```python
from build123d import *

# Parameters (mm, degrees)
SKETCH1_R                = 50
BOSS_EXTRUDE1_DEPTH      = 5
SKETCH2_R                = 15
BOSS_EXTRUDE2_DEPTH      = 5
SKETCH3_R                = 9
CUT_EXTRUDE1_DEPTH       = 15
BOSS_EXTRUDE3_REACH      = 118.726
BOSS_EXTRUDE3_END_RADIUS = 50
SKETCH6_R                = 1.25
BOSS_EXTRUDE4_DEPTH      = 5
CIRPATTERN3_COUNT        = 4


with BuildPart() as part:
    # Sketch1 → Boss-Extrude1 (new body)
    with BuildSketch(Plane.XY):
        Circle(SKETCH1_R)
    extrude(amount=BOSS_EXTRUDE1_DEPTH)

    # Sketch2 → Boss-Extrude2 (add)
    with BuildSketch(Plane.XY.offset(5)):
        Circle(SKETCH2_R)
    extrude(amount=BOSS_EXTRUDE2_DEPTH)

    # Sketch3 → Cut-Extrude1 (cut)
    with BuildSketch(Plane.XY.offset(10)):
        Circle(SKETCH3_R)
    extrude(amount=-CUT_EXTRUDE1_DEPTH, mode=Mode.SUBTRACT)

    # Boss-Extrude3: up to this cylinder (the profile starts outside it)
    boss_extrude3_end = Plane(origin=(0, 0, 2.5), z_dir=(0, 0, -1)) * Cylinder(BOSS_EXTRUDE3_END_RADIUS, 338.452, mode=Mode.PRIVATE)
    # Sketch4 → Boss-Extrude3 (add, up to the surface)
    with BuildSketch(Plane(origin=(0, 55, 0), x_dir=(1, 0, 0), z_dir=(0, 1, 0)), mode=Mode.PRIVATE) as boss_extrude3_sk1:
        Polygon((0, 0), (2.5, 0), (2.5, -5), (-2.5, -5), (-2.5, 0), align=None)
    boss_extrude3_tool1 = extrude(boss_extrude3_sk1.sketch, amount=-BOSS_EXTRUDE3_REACH, mode=Mode.PRIVATE) - boss_extrude3_end
    boss_extrude3 = boss_extrude3_tool1.solids().sort_by_distance((0, 55, 2.5))[0]
    add(boss_extrude3)

    # Sketch6 → Boss-Extrude4 (add, symmetric)
    with BuildSketch(Plane(origin=(0, 0, 0), x_dir=(0, 0, -1), z_dir=(1, 0, 0))):
        with Locations(Location((-2.5, 52.8, 0), (0, 0, 180))):
            Circle(SKETCH6_R)
    boss_extrude4 = extrude(amount=BOSS_EXTRUDE4_DEPTH, both=True)

    # CirPattern3: Boss-Extrude3, Boss-Extrude4 ×4 about axis
    cirpattern3_axis = Axis((0, 0, 0), (0, 0, 1))
    add([boss_extrude3.rotate(cirpattern3_axis, i * 360 / CIRPATTERN3_COUNT) for i in range(1, CIRPATTERN3_COUNT)])
    add([boss_extrude4.rotate(cirpattern3_axis, i * 360 / CIRPATTERN3_COUNT) for i in range(1, CIRPATTERN3_COUNT)])


solid = part.part
```
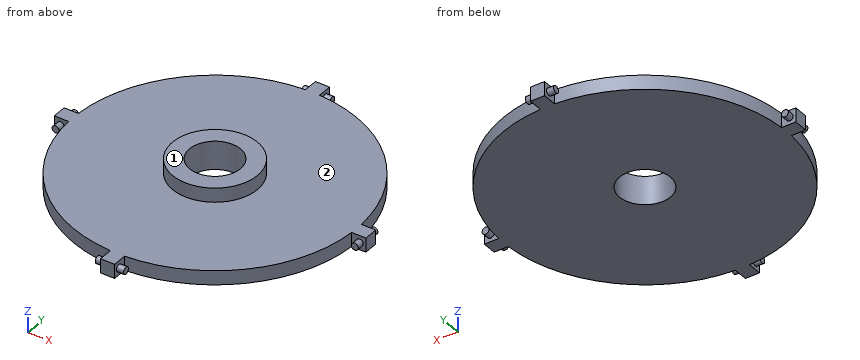
Verification items for the finished model (mm, model axes). Face numbers are marked on the shaded views. A direction names the side the tool comes from. Round coordinates to 2 decimals unless told otherwise and drop trailing zeros. Write each loop counter-clockwise with the first axis right and the second up, starting at its lowest first coordinate (ties: lowest second). Pieces come first, ordered by that corner, then holes.
1. Section check C-C on x = 52.8. Enter the section's corners in (y, z).
2. Section check A-A on y = 0. Enter the section's corners in (x, z), plus the area to 3 significant figures.
3. Section check D-D on z = 8.5. Enter the section's corners in (x, y).
4. Access from +Z, -Z, +X, -X, +Y, -Y to the whole of each face (thin tool, end or side, straight path). Record for the marked faces 1 and 2.
5. Scan lines: L1, parallel to Y at x = 0, z = 7.5; L2, parallel to Y at x = 50.5, z = 3.25; L3, parallel to X at y = -1, z = 9.75. Record each from-to range of solid material in increasing order.
6. Gauge pin test, flat ends, axial feed: P1, Ø1, axis at x = -37.5, y = 7, coming from the -Z side; P2, Ø2, axis at y = 53, z = 2.5, coming from the +X side; P3, Ø2.5, axis at x = -52.5, z = 2, coming from the +Y side; P4, Ø1.5, axis at y = 53.5, z = 2.5, coming from the -X side. Record the tip position at first contact, or that the pin passes through.
Answer:
1. outline: (-5, 1.25) - (-2.5, 1.25) - (-2.5, 0) - (2.5, 0) - (2.5, 1.25) - (5, 1.25) - (5, 3.75) - (2.5, 3.75) - (2.5, 5) - (-2.5, 5) - (-2.5, 3.75) - (-5, 3.75) - close
2. outline: (-55, 0) - (-9, 0) - (-9, 10) - (-15, 10) - (-15, 5) - (-55, 5) - close; (9, 0) - (55, 0) - (55, 5) - (15, 5) - (15, 10) - (9, 10) - close
2. area: 520 mm2
3. outline: circle Ø30 at (0, 0); hole circle Ø18 at (0, 0)
4. face 1: +Z, +X, -X, +Y, -Y
4. face 2: +Z
5. L1: y = -15 to -9, 9 to 15
5. L2: y = -2.5 to 2.5
5. L3: x = -14.97 to -8.94, 8.94 to 14.97
6. P1: stops at z = 0
6. P2: stops at x = 5
6. P3: stops at y = 5
6. P4: stops at x = -5
